Here's how the part is built. I have some questions about the finished solid (model axes, mm). A direction names the side the tool comes from. Give positions to 0.01 mm unless a question says otherwise; leave off trailing zeros. Loops run counter-clockwise (first coordinate to the right, second up) from the corner with the lowest first, then second, coordinate; pieces in that order, holes last. Notation, with made-up numbers: (61, 29) -> (81, 29) arc R27 ccw to (81, 57) -> close; hole circle Ø3 at (53.5, 60.5). An arc over 180 degrees is marked (long way). Answer in a Markdown table with one row per item. Add a question column.
Item 1: If we section it at D-D (z = -2.5): Write out the boundary of the cut face in (x, y), then the cut area to 3 significant figures.
Item 2: For P1, Ø1, axis at x = 9.5, z = 3, coming from the +Y side; P2, Ø3, axis at y = -2.5, z = -1, coming from the +X side; P3, Ø1, axis at x = -2, z = 1.5, coming from the +Y side, each with a flat end and sliding along its axis, tell me the tip position at first contact or that it passes through.
Item 3: We'd pull the mould along Z, two halves only. Please class faces 4 (the face through (-2, -3, -4)), 5 (the face through (-7, -7.5, 1)), 6 (the face through (-14.669, -5.035, -0.526)), 7 (the face through (-3.25, -5.03, -0.08)): released by +Z, released by -Z, zero draft, split by the parting line, or undercut.
Item 4: If I drill on line 1 (Z direction, x = -5, y = -3.6); line 2 (X direction, y = -3.25, z = 0.5); line 3 (Y direction, x = 11.5, z = -1), over which ranges is the centre line in solid material (lowest first)?
Item 5: Which directions (+Z, -Z, +X, -X, +Y, -Y) give clear straight access to the entire face, cutting with the end or side of a thin tool? Please do faces 1 (the face through (-8, -2.5, 0)), 2 (the face through (5, -2, 0)), 3 (the face through (-2, -3, 4)).
Item 6: If we section it at B-B (z = 0): Write out the boundary of the cut face in (x, y).
Item 7: If we section it at C-C (y = -6): Write out the boundary of the cut face in (x, z).
Item 8: If we section it at A-A (x = -5): Write out the boundary of the cut face in (y, z), then the cut area to 3 significant figures.
```python
from build123d import *

# Parameters (mm, degrees)
SKETCH1_W                  = 32
SKETCH1_H                  = 15
BOSS_EXTRUDE1_DEPTH        = 4
SKETCH2_W                  = 16
SKETCH2_H                  = 10
SKETCH2_W_2                = 11
CUT_EXTRUDE1_DEPTH         = 20.397164741
CHAMFER1_SIZE              = 1
CHAMFER2_SIZE              = 2
F_3_5_3_5_DIAMETER_HOLE1_D = 3.5
CHAMFER3_SIZE              = 3
CHAMFER3_SIZE2             = 10
CHAMFER4_SIZE              = 10
CHAMFER4_SIZE2             = 3


with BuildPart() as part:
    # Sketch1 → Boss-Extrude1 (new, symmetric)
    with BuildSketch(Plane.XY):
        Rectangle(SKETCH1_W, SKETCH1_H)
    extrude(amount=BOSS_EXTRUDE1_DEPTH, both=True)

    # Sketch2 → Cut-Extrude1 (cut, through all)
    with BuildSketch(Plane.XY.offset(4)):
        with Locations((-8, 2.5)):
            Rectangle(SKETCH2_W, SKETCH2_H)
        with Locations((10.5, -2.5)):
            Rectangle(SKETCH2_W_2, SKETCH2_H)
    extrude(amount=-CUT_EXTRUDE1_DEPTH, mode=Mode.SUBTRACT)

    # Chamfer1
    chamfer1_edges = [part.edges().sort_by_distance(p)[0] for p in [
        (-16, -5, -4),
        (-16, -5, 4),
    ]]
    chamfer(chamfer1_edges, length=CHAMFER1_SIZE)

    # Chamfer2
    chamfer2_edges = [part.edges().sort_by_distance(p)[0] for p in [
        (0, 7.5, 0),
        (5, -7.5, 0),
    ]]
    chamfer(chamfer2_edges, length=CHAMFER2_SIZE)

    # Ø3.5 (3.5) Diameter Hole1 (through all)
    with Locations(Plane(origin=(0, -2.5, 0), x_dir=(1, 0, 0), z_dir=(0, 1, 0))):
        with Locations((-13, 0), (-5, 0)):
            Hole(F_3_5_3_5_DIAMETER_HOLE1_D / 2)

    # Chamfer3
    chamfer3_edges = [part.edges().sort_by_distance(p)[0] for p in [
        (16, 5, 4),
    ]]
    chamfer3_side = [part.faces().sort_by_distance(p)[0] for p in [
        (16, 5, 0),
    ]]
    chamfer(chamfer3_edges, length=CHAMFER3_SIZE, length2=CHAMFER3_SIZE2, reference=chamfer3_side[0])

    # Chamfer4
    chamfer4_edges = [part.edges().sort_by_distance(p)[0] for p in [
        (16, 5, -4),
    ]]
    chamfer4_side = [part.faces().sort_by_distance(p)[0] for p in [
        (0.957711443, -0.497512438, -4),
    ]]
    chamfer(chamfer4_edges, length=CHAMFER4_SIZE, length2=CHAMFER4_SIZE2, reference=chamfer4_side[0])


solid = part.part
```
Recorded:
| question | item | result |
|---|---|---|
| 1 | outline | (-16, -7.5) -> (3, -7.5) -> (5, -5.5) -> (5, 2.5) -> (11, 2.5) -> (11, 7.5) -> (2, 7.5) -> (0, 5.5) -> (0, -2.5) -> (-16, -2.5) -> close |
| 1 | area | 181 mm^2 |
| 2 | P1 | stops at y = 7.5 |
| 2 | P2 | stops at x = 5 |
| 2 | P3 | stops at y = -2.5 |
| 3 | face 4 | released by -Z |
| 3 | face 5 | zero draft |
| 3 | face 6 | undercut |
| 3 | face 7 | undercut |
| 4 | line 1 | z = -4 to -1.75, 1.75 to 4 |
| 4 | line 2 | x = -16 to -14.68, -11.32 to -6.68, -3.32 to 5 |
| 4 | line 3 | y = 2.5 to 7.5 |
| 5 | face 1 | +Z, -Z, -X, +Y |
| 5 | face 2 | +Z, -Z, +X, -Y |
| 5 | face 3 | +Z, +X, -X, +Y, -Y |
| 6 | outline | (-16, -7.5) -> (-14.75, -7.5) -> (-14.75, -2.5) -> (-16, -2.5) -> close; (-11.25, -7.5) -> (-6.75, -7.5) -> (-6.75, -2.5) -> (-11.25, -2.5) -> close; (-3.25, -7.5) -> (3, -7.5) -> (5, -5.5) -> (5, 2.5) -> (16, 2.5) -> (16, 7.5) -> (2, 7.5) -> (0, 5.5) -> (0, -2.5) -> (-3.25, -2.5) -> close |
| 7 | outline | (-16, -3) -> (-15, -4) -> (4.5, -4) -> (4.5, 4) -> (-15, 4) -> (-16, 3) -> close; hole circle Ø3.5 at (-13, 0); hole circle Ø3.5 at (-5, 0) |
| 8 | outline | (-7.5, -4) -> (-2.5, -4) -> (-2.5, -1.75) -> (-7.5, -1.75) -> close; (-7.5, 1.75) -> (-2.5, 1.75) -> (-2.5, 4) -> (-7.5, 4) -> close |
| 8 | area | 22.5 mm^2 |
